For this review, take the finished solid that the model builds, in its own axes (mm). A direction names the side the tool comes from. Coordinates: 2 decimals unless noted, no trailing zeros. Write each loop counter-clockwise with the first axis right and the second up, starting at its lowest first coordinate (ties: lowest second). Pieces come first, ordered by that corner, then holes. Notation, with made-up numbers: (35, 89) - (78, 89) arc R24 cw to (78, 106) - close; hole circle Ø3 at (20, 36.25). An arc over 180 degrees is marked (long way). Write each question's results on one line, items separated by ' | '.
from build123d import *

# Parameters (mm, degrees)
BOSS_EXTRUDE1_DEPTH = 20
CUT_EXTRUDE1_DEPTH  = 308.44105126


with BuildPart() as part:
    # Sketch1 → Boss-Extrude1 (new body)
    with BuildSketch(Plane.XY):
        with BuildLine():
            Line((45, 188), (45, 70))
            ThreePointArc((45, 70), (39.142135624, 55.857864376), (25, 50))
            Line((25, 50), (5, 50))
            Line((5, 50), (0, 45))
            Line((0, 45), (0, 5))
            Line((0, 5), (5, 0))
            Line((5, 0), (161, 0))
            Line((161, 0), (166, 5))
            Line((166, 5), (166, 253))
            Line((166, 253), (161, 258))
            Line((161, 258), (5, 258))
            Line((5, 258), (0, 253))
            Line((0, 253), (0, 213))
            Line((0, 213), (5, 208))
            Line((5, 208), (25, 208))
            ThreePointArc((25, 208), (39.142135624, 202.142135624), (45, 188))
        make_face()
    extrude(amount=BOSS_EXTRUDE1_DEPTH)

    # Sketch2 → Cut-Extrude1 (cut, through all)
    with BuildSketch(Plane.XZ):
        Polygon((0, 20), (0, 0), (9, 0), align=None)
        Polygon((166, 20), (166, 0), (144, 0), align=None)
    extrude(amount=-CUT_EXTRUDE1_DEPTH, mode=Mode.SUBTRACT)


solid = part.part
Q1. Wall thickness on line 1 along Y through (x, z) = (25, 8); line 2 along Y through (x, z) = (40.5, 13.75); line 3 along X through (y, z) = (39.5, 3): over which ranges is each line inside the solid? List them lowest first. Write a range as from..to.
Results found:
line 1: 0..50, 208..258 | line 2: 0..57.36, 200.64..258 | line 3: 7.65..147.3
Q2. For pin 1 (8 mm diameter, centred on x = 127, z = 3.5, fed in from -Y); pin 2 (5 mm diameter, centred on y = 230, z = 2.5, fed in from +X); pin 3 (3 mm diameter, centred on y = 49, z = 11.5, fed in from +X); pin 4 (6 mm diameter, centred on y = 135.5, z = 10.5, fed in from -X), all flat-tipped, find the tip position at first contact; note any pin that passes through.
Results found:
pin 1: y = 0 | pin 2: x = 149.5 | pin 3: x = 158.3 | pin 4: x = 45
Q3. Take a section at A-A on x = 13. State the section outline as (y, z) points, plus the area to 3 significant figures.
Results found:
outline: (0, 0) - (50, 0) - (50, 20) - (0, 20) - close; (208, 0) - (258, 0) - (258, 20) - (208, 20) - close | area: 2,000 mm2
Q4. Take a section at D-D on y = 57.5. State the section outline as (x, z) points.
Results found:
outline: (40.61, 0) - (144, 0) - (166, 20) - (40.61, 20) - close
Q5. For faces 4 (the face through (45, 130, 10)), 5 (the face through (155, 127, 10)), list the 3-axis set-ups (+Z, -Z, +X, -X, +Y, -Y) from which the entire face can be reached by the end or side of a thin tool; tool diameter is ignored.
Results found:
face 4: +Z, -Z, -X | face 5: -Z, +X, +Y, -Y
Q6. Take a section at B-B on z = 12. State the section outline as (x, y) points, plus the area to 3 significant figures.
Results found:
outline: (3.6, 1.4) - (5, 0) - (157.2, 0) - (157.2, 258) - (5, 258) - (3.6, 256.6) - (3.6, 209.4) - (5, 208) - (25, 208) arc R20 cw to (45, 188) - (45, 70) arc R20 cw to (25, 50) - (5, 50) - (3.6, 48.6) - close | area: 33,300 mm2
Q7. Take a section at C-C on y = 137. State the section outline as (x, z) points, plus the area to 3 significant figures.
Results found:
outline: (45, 0) - (144, 0) - (166, 20) - (45, 20) - close | area: 2,200 mm2
Q8. Mouldability with a two-part tool opening along Y and no side actions: class faces 1 (the face through (15, 50, 10)), 2 (the face through (162, 257, 19)), 3 (the face through (82, 0, 10)) as pulls with the +Y half, pulls with the -Y half, needs draft (parallel to the pull), parting line crosses it, or undercut.
Results found:
face 1: undercut | face 2: pulls with the +Y half | face 3: pulls with the -Y half
